Can you work these out from the model? Positions are in its coordinate system, mm. A direction names the side the tool comes from. Give positions to 0.01 mm unless a question says otherwise; leave off trailing zeros. Order: outer loops, then holes, each group sorted by start corner. A loop starts at its lowest first (then second) coordinate and runs counter-clockwise, first axis right, second up. Notation, with made-up numbers: M 40,20 L 84,20 A14 cw 84,27 Z; hole C -15.5,35.25 d11. An arc over 180 degrees is marked long. Use one line per item in the form item = value. Start each with the question number.
1. Will these pins go through, and if not, where does the flat tip stop? P1, Ø3, axis at x = 7.5, z = 3, coming from the -Y side; P2, Ø5.5, axis at x = -5, y = 7.5, coming from the -Z side; P3, Ø2.5, axis at x = 10, z = 4, coming from the +Y side.
2. We'd pull the mould along Z, two halves only. Please class faces 1 (the face through (-22, 0.5, 0.2)), 2 (the face through (0, 7, 13)), 3 (the face through (8.06, 7.9, 4.8)): +Z half, -Z half, draft (parallel to the pull), parting line (faces both ways), or undercut.
3. I want a section at C-C, the plane y = 12.25. List the corners of the cut face in (x, z) for me, and give its area (3 significant figures).
4. I want a section at B-B, the plane z = 0.25. List the corners of the cut face in (x, y) for me.
5. For faces 4 (the face through (-15, 4, 6.2)), 5 (the face through (22, 0.5, 0.2)), 6 (the face through (2, 7.6, -7.9)), which set-ups out of +Z, -Z, +X, -X, +Y, -Y let a thin tool reach every point of the face, with its end or its side?
6. I need wall thicknesses on L1, parallel to Y at x = 15, z = 11.75; L2, parallel to Y at x = -15, z = -5.25; L3, parallel to X at y = 3.25, z = 10.75. Which ranges of each line are inside material? Lowest first, please.
7. I want a section at A-A, the plane x = 15. List the corners of the cut face in (y, z) for me, and give its area (3 significant figures).
8. I want a section at D-D, the plane z = -9.5. List the corners of the cut face in (x, y) for me.
```python
from build123d import *

# Parameters (mm, degrees)
SKETCH1_W                                            = 45
SKETCH1_H                                            = 26
BOSS_EXTRUDE1_DEPTH                                  = 15
SKETCH2_R                                            = 5
CUT_EXTRUDE1_DEPTH                                   = 31.004166377
F_6_0MM_DOWEL_HOLE_1_D                               = 6
F_6_0MM_DOWEL_HOLE_1_DEPTH                           = 10
F_6_0MM_DOWEL_HOLE_1_TIP                             = 1.802581857
CHAMFER1_SIZE                                        = 1
CBORE_FOR_M6_HEXAGON_SOCKET_HEAD_CAP_SCR_D           = 6.6
CBORE_FOR_M6_HEXAGON_SOCKET_HEAD_CAP_SCR_CBORE_D     = 11
CBORE_FOR_M6_HEXAGON_SOCKET_HEAD_CAP_SCR_CBORE_DEPTH = 6.8
M5_TAPPED_HOLE1_D                                    = 4.2
M5_TAPPED_HOLE1_DEPTH                                = 14
M5_TAPPED_HOLE1_TIP                                  = 1.2618073


with BuildPart() as part:
    # Sketch1 → Boss-Extrude1 (new body)
    with BuildSketch(Plane(origin=(0, 0, 0), x_dir=(1, 0, 0), z_dir=(0, 1, 0))):
        Rectangle(SKETCH1_W, SKETCH1_H)
    extrude(amount=BOSS_EXTRUDE1_DEPTH)

    # Sketch2 → Cut-Extrude1 (cut, through all)
    with BuildSketch(Plane(origin=(0, 15, 0), x_dir=(1, 0, 0), z_dir=(0, 1, 0))):
        with Locations(Location((0, -4, 0), (0, 0, 270))):
            Circle(SKETCH2_R)
    extrude(amount=-CUT_EXTRUDE1_DEPTH, mode=Mode.SUBTRACT)

    # Ø6.0mm Dowel Hole 1
    with Locations(Plane(origin=(0, 0, -13), x_dir=(-1, 0, 0), z_dir=(0, 0, -1))):
        with Locations((-5, 7.5), (5, 7.5)):
            Hole(F_6_0MM_DOWEL_HOLE_1_D / 2, depth=F_6_0MM_DOWEL_HOLE_1_DEPTH)
            with Locations((0, 0, -(F_6_0MM_DOWEL_HOLE_1_DEPTH + F_6_0MM_DOWEL_HOLE_1_TIP / 2))):  # 118° drill point
                Cone(0, F_6_0MM_DOWEL_HOLE_1_D / 2, F_6_0MM_DOWEL_HOLE_1_TIP, mode=Mode.SUBTRACT)

    # Chamfer1
    chamfer1_edges = [part.edges().sort_by_distance(p)[0] for p in [
        (-22.5, 15, 0),
        (22.5, 15, 0),
        (-22.5, 0, 0),
        (22.5, 0, 0),
    ]]
    chamfer(chamfer1_edges, length=CHAMFER1_SIZE)

    # CBORE for M6 Hexagon socket head cap screws1 (through all)
    with Locations(Plane.XY.offset(13)):
        with Locations((-15, 7.5), (15, 7.5)):
            CounterBoreHole(CBORE_FOR_M6_HEXAGON_SOCKET_HEAD_CAP_SCR_D / 2, CBORE_FOR_M6_HEXAGON_SOCKET_HEAD_CAP_SCR_CBORE_D / 2, CBORE_FOR_M6_HEXAGON_SOCKET_HEAD_CAP_SCR_CBORE_DEPTH)

    # M5 Tapped Hole1
    with Locations(Plane(origin=(0, 15, 0), x_dir=(1, 0, 0), z_dir=(0, 1, 0))):
        with Locations((10, -4)):
            Hole(M5_TAPPED_HOLE1_D / 2, depth=M5_TAPPED_HOLE1_DEPTH)
            with Locations((0, 0, -(M5_TAPPED_HOLE1_DEPTH + M5_TAPPED_HOLE1_TIP / 2))):  # 118° drill point
                Cone(0, M5_TAPPED_HOLE1_D / 2, M5_TAPPED_HOLE1_TIP, mode=Mode.SUBTRACT)


solid = part.part
```
Check result:
q1.P1 = 0
q1.P2 = -2.85
q1.P3 = 0.49
q2.face_1 = draft
q2.face_2 = +Z half
q2.face_3 = undercut
q3.outline = M -22.5,-13 L 22.5,-13 L 22.5,13 L 17.77,13 L 17.77,6.2 L 12.23,6.2 L 12.23,13 L -12.23,13 L -12.23,6.2 L -17.77,6.2 L -17.77,13 L -22.5,13 Z; hole C 0,4 d10; hole C 10,4 d4.2
q3.area = 1,000 mm2
q4.outline = M -22.5,1 L -21.5,0 L -3.31,0 L -3.31,15 L -21.5,15 L -22.5,14 Z; M 3.31,0 L 21.5,0 L 22.5,1 L 22.5,14 L 21.5,15 L 3.31,15 Z; hole C -15,7.5 d6.6; hole C 15,7.5 d6.6
q5.face_4 = +Z
q5.face_5 = +Z, -Z, +X, -Y
q5.face_6 = -Z
q6.L1 = 0 to 2, 13 to 15
q6.L2 = 0 to 4.2, 10.8 to 15
q6.L3 = -22.5 to -18.49, -11.51 to 11.51, 18.49 to 22.5
q7.outline = M 0,-13 L 4.2,-13 L 4.2,6.2 L 2,6.2 L 2,13 L 0,13 Z; M 10.8,-13 L 15,-13 L 15,13 L 13,13 L 13,6.2 L 10.8,6.2 Z
q7.area = 188 mm2
q8.outline = M -22.5,1 L -21.5,0 L 21.5,0 L 22.5,1 L 22.5,14 L 21.5,15 L -21.5,15 L -22.5,14 Z; hole C -15,7.5 d6.6; hole C -5,7.5 d6; hole C 5,7.5 d6; hole C 15,7.5 d6.6
